Build history of the part. All positions in model axes, mm. A direction names the side the tool comes from. Give positions to 0.01 mm unless a question says otherwise; leave off trailing zeros. Write each loop counter-clockwise with the first axis right and the second up, starting at its lowest first coordinate (ties: lowest second). Pieces come first, ordered by that corner, then holes. Notation, with made-up numbers: (0.5, 32.25) -> (12.5, 32.25) arc R13 cw to (12.5, 50.25) -> close; hole circle Ø4 at (46, 66.25). An arc over 180 degrees is marked (long way). Write item = value, one per line. Start each with the question number.
Q1. Tool access for faces 5 (the face through (-5, -5, 3)), 6 (the face through (0.33, -1.486, -7.493)), 7 (the face through (-2, -15, -4)): list every direction of +Z, -Z, +X, -X, +Y, -Y with a clear straight run to the whole face (end or side of a thin tool).
Q2. Saw through at B-B, the plane y = -12.25. List the corners of the cut face in (x, z).
Q3. Wall check: line 1 (X direction, y = -12, z = 0); line 2 (Y direction, x = 0.75, z = 6.75); line 3 (Y direction, x = 0.5, z = 4.5). Give the ranges that are in metal, low to high.
Q4. Saw through at A-A, the plane y = -21.25. List the corners of the cut face in (x, z).
Q5. Mould opens along Y. For faces 1 (the face through (-1, 0, 3)), 2 (the face through (-5.37, -3.99, -1.19)), 3 (the face through (-3, -20, 0)), 4 (the face through (1.802, -9.683, 5.723)) say: pulls with the +Y half, pulls with the -Y half, needs draft (parallel to the pull), parting line crosses it, or undercut.
Q6. Drop flat-ended pins along their axis: P1, Ø8, axis at y = -14.5, z = 2.5, coming from the +X side; P2, Ø2, axis at x = 3, z = -3, coming from the -Y side; P3, Ø5, axis at x = 5, y = -12.5, coming from the +Z side. Give the stop position or say it passes through.
from build123d import *

# Parameters (mm, degrees)
SKETCH_1_R          = 6
EXTRUDE_1_DEPTH     = 15
SKETCH_2_R          = 2.5
EXTRUDE_2_DEPTH     = 15
SKETCH_3_R          = 2
CUT_EXTRUDE_1_DEPTH = 32.176914536
CHAMFER_2_SIZE      = 0.5
SKETCH_6_R          = 7.5
SKETCH_6_R_2        = 6
EXTRUDE_3_DEPTH     = 3
CHAMFER_3_SIZE      = 1
CHAMFER_4_SIZE      = 0.5
SKETCH_7_R          = 4
SKETCH_7_R_2        = 2.5
EXTRUDE_4_DEPTH     = 5
CHAMFER_5_SIZE      = 0.3
CHAMFER_6_SIZE      = 0.3
SKETCH_8_W          = 3.367745964
SKETCH_8_H          = 2


with BuildPart() as part:
    # 草图1 → 凸台-拉伸1 (new body)
    with BuildSketch(Plane(origin=(0, 0, 0), x_dir=(1, 0, 0), z_dir=(0, 1, 0))):
        with Locations(Location((0, 0, 0), (0, 0, 270))):
            Circle(SKETCH_1_R)
    extrude(amount=-EXTRUDE_1_DEPTH)

    # 草图2 → 凸台-拉伸2 (add)
    with BuildSketch(Plane.XZ.offset(15)):
        with Locations(Location((0, 0, 0), (0, 0, 90))):
            Circle(SKETCH_2_R)
    extrude(amount=EXTRUDE_2_DEPTH)

    # 草图3 → 切除-拉伸1 (cut, through all)
    with BuildSketch(Plane(origin=(0, 0, 0), x_dir=(1, 0, 0), z_dir=(0, 1, 0))):
        with Locations(Location((0, 0, 0), (0, 0, 270))):
            Circle(SKETCH_3_R)
    extrude(amount=-CUT_EXTRUDE_1_DEPTH, mode=Mode.SUBTRACT)

    # 倒角2
    chamfer_2_edges = [part.edges().sort_by_distance(p)[0] for p in [
        (0, -15, -6),
    ]]
    chamfer(chamfer_2_edges, length=CHAMFER_2_SIZE)

    # 草图6 → 凸台-拉伸3 (add)
    with BuildSketch(Plane(origin=(0, 0, 0), x_dir=(1, 0, 0), z_dir=(0, 1, 0))):
        with Locations(Location((0, 0, 0), (0, 0, 270))):
            Circle(SKETCH_6_R)
        with Locations(Location((0, 0, 0), (0, 0, 270))):
            Circle(SKETCH_6_R_2, mode=Mode.SUBTRACT)
    extrude(amount=-EXTRUDE_3_DEPTH)

    # 倒角3
    chamfer_3_edges = [part.edges().sort_by_distance(p)[0] for p in [
        (0, 0, -2),
    ]]
    chamfer(chamfer_3_edges, length=CHAMFER_3_SIZE)

    # 倒角4
    chamfer_4_edges = [part.edges().sort_by_distance(p)[0] for p in [
        (0, -3, -7.5),
        (0, 0, -7.5),
    ]]
    chamfer(chamfer_4_edges, length=CHAMFER_4_SIZE)

    # 草图7 → 凸台-拉伸4 (add)
    with BuildSketch(Plane.XZ.offset(15)):
        with Locations(Location((0, 0, 0), (0, 0, 90))):
            Circle(SKETCH_7_R)
        with Locations(Location((0, 0, 0), (0, 0, 270))):
            Circle(SKETCH_7_R_2, mode=Mode.SUBTRACT)
    extrude(amount=EXTRUDE_4_DEPTH)

    # 倒角5
    chamfer_5_edges = [part.edges().sort_by_distance(p)[0] for p in [
        (0, -20, -4),
    ]]
    chamfer(chamfer_5_edges, length=CHAMFER_5_SIZE)

    # 倒角6
    chamfer_6_edges = [part.edges().sort_by_distance(p)[0] for p in [
        (0, -30, -2.5),
    ]]
    chamfer(chamfer_6_edges, length=CHAMFER_6_SIZE)

    # 草图8 → 切除-旋转1 (revolve, cut)
    with BuildSketch(Plane.XY, mode=Mode.PRIVATE) as cut_revolve_1_sk:
        with Locations((-7.183872982, -4)):
            Rectangle(SKETCH_8_W, SKETCH_8_H)
    revolve(cut_revolve_1_sk.sketch.rotate(Axis((0, -15, 0), (0, 1, 0)), 90), axis=Axis((0, -15, 0), (0, 1, 0)), mode=Mode.SUBTRACT)


solid = part.part
Report:
q1.face_5 = none
q1.face_6 = +Y, -Y
q1.face_7 = -Y
q2.outline = circle Ø12 at (0, 0); hole circle Ø4 at (0, 0)
q3.line_1 = -6 to -2, 2 to 6
q3.line_2 = -3 to 0
q3.line_3 = -15 to 0
q4.outline = circle Ø5 at (0, 0); hole circle Ø4 at (0, 0)
q5.face_1 = pulls with the +Y half
q5.face_2 = undercut
q5.face_3 = pulls with the -Y half
q5.face_4 = needs draft
q6.P1 = 6
q6.P2 = -20
q6.P3 = 5.45
